For this review, take the finished solid that the model builds, in its own axes (mm). Give positions to 0.01 mm unless a question says otherwise; leave off trailing zeros. Loops run counter-clockwise (first coordinate to the right, second up) from the corner with the lowest first, then second, coordinate; pieces in that order, holes last.
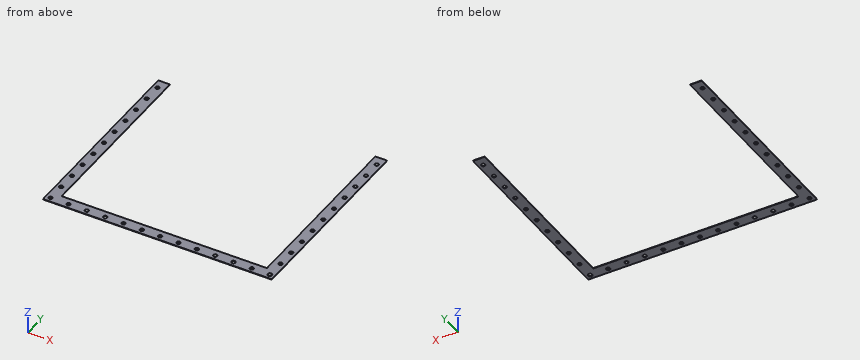
```python
from build123d import *

# Parameters (mm, degrees)
SKETCH1_R           = 12
SKETCH1_R_2         = 13.848900056
BOSS_EXTRUDE1_DEPTH = 3


with BuildPart() as part:
    # Sketch1 → Boss-Extrude1 (new body)
    # profile 1 of 2: a face of its own
    with BuildSketch(Plane.XY):
        with BuildLine():
            Line((7.821297611, 64.305720246), (-66.178702389, 64.305720246))
            Line((-66.178702389, 64.305720246), (-66.178702389, -1185.694279754))
            Line((-66.178702389, -1185.694279754), (657.821297611, -1185.694279754))
            Line((657.821297611, -1185.694279754), (657.821297611, -1167.694279754))
            ThreePointArc((657.821297611, -1167.694279754), (645.821297611, -1155.694279754), (657.821297611, -1143.694279754))
            Line((657.821297611, -1143.694279754), (657.821297611, -1111.694279754))
            Line((657.821297611, -1111.694279754), (7.821297611, -1111.694279754))
            Line((7.821297611, -1111.694279754), (7.821297611, 64.305720246))
        make_face()
        with Locations((-36.178702389, -1155.694279754)):
            Circle(SKETCH1_R, mode=Mode.SUBTRACT)
        with Locations((77.821297611, -1155.694279754)):
            Circle(SKETCH1_R, mode=Mode.SUBTRACT)
        with Locations((-36.178702389, -1039.694279754)):
            Circle(SKETCH1_R, mode=Mode.SUBTRACT)
        with Locations((193.821297611, -1155.694279754)):
            Circle(SKETCH1_R, mode=Mode.SUBTRACT)
        with Locations((-36.178702389, -923.694279754)):
            Circle(SKETCH1_R, mode=Mode.SUBTRACT)
        with Locations((309.821297611, -1155.694279754)):
            Circle(SKETCH1_R, mode=Mode.SUBTRACT)
        with Locations((425.821297611, -1155.694279754)):
            Circle(SKETCH1_R, mode=Mode.SUBTRACT)
        with Locations((541.821297611, -1155.694279754)):
            Circle(SKETCH1_R, mode=Mode.SUBTRACT)
        with Locations((-36.178702389, -807.694279754)):
            Circle(SKETCH1_R, mode=Mode.SUBTRACT)
        with Locations((-36.178702389, -691.694279754)):
            Circle(SKETCH1_R, mode=Mode.SUBTRACT)
        with Locations((-36.178702389, -575.694279754)):
            Circle(SKETCH1_R, mode=Mode.SUBTRACT)
        with Locations((-36.178702389, -459.694279754)):
            Circle(SKETCH1_R, mode=Mode.SUBTRACT)
        with Locations((-36.178702389, -343.694279754)):
            Circle(SKETCH1_R, mode=Mode.SUBTRACT)
        with Locations((-36.178702389, -227.694279754)):
            Circle(SKETCH1_R, mode=Mode.SUBTRACT)
        with Locations((-36.178702389, -111.694279754)):
            Circle(SKETCH1_R, mode=Mode.SUBTRACT)
        with Locations((-36.178702389, 4.305720246)):
            Circle(SKETCH1_R, mode=Mode.SUBTRACT)
    # profile 2 of 2: a face of its own
    with BuildSketch(Plane.XY):
        with BuildLine():
            Line((657.821297611, -1167.694279754), (657.821297611, -1185.694279754))
            Line((657.821297611, -1185.694279754), (1381.821297611, -1185.694279754))
            Line((1381.821297611, -1185.694279754), (1381.821297611, 64.305720246))
            Line((1381.821297611, 64.305720246), (1307.821297611, 64.305720246))
            Line((1307.821297611, 64.305720246), (1307.821297611, -1111.694279754))
            Line((1307.821297611, -1111.694279754), (657.821297611, -1111.694279754))
            Line((657.821297611, -1111.694279754), (657.821297611, -1143.694279754))
            ThreePointArc((657.821297611, -1143.694279754), (666.306578985, -1147.20899838), (669.821297611, -1155.694279754))
            ThreePointArc((669.821297611, -1155.694279754), (666.306578985, -1164.179561128), (657.821297611, -1167.694279754))
        make_face()
        with Locations((773.821297611, -1155.694279754)):
            Circle(SKETCH1_R, mode=Mode.SUBTRACT)
        with Locations((889.821297611, -1155.694279754)):
            Circle(SKETCH1_R, mode=Mode.SUBTRACT)
        with Locations((1005.821297611, -1155.694279754)):
            Circle(SKETCH1_R, mode=Mode.SUBTRACT)
        with Locations((1121.821297611, -1155.694279754)):
            Circle(SKETCH1_R, mode=Mode.SUBTRACT)
        with Locations((1237.821297611, -1155.694279754)):
            Circle(SKETCH1_R, mode=Mode.SUBTRACT)
        with Locations((1351.821297611, -1155.694279754)):
            Circle(SKETCH1_R_2, mode=Mode.SUBTRACT)
        with Locations((1351.821297611, -1039.694279754)):
            Circle(SKETCH1_R, mode=Mode.SUBTRACT)
        with Locations((1351.821297611, -923.694279754)):
            Circle(SKETCH1_R, mode=Mode.SUBTRACT)
        with Locations((1351.821297611, -807.694279754)):
            Circle(SKETCH1_R, mode=Mode.SUBTRACT)
        with Locations((1351.821297611, -691.694279754)):
            Circle(SKETCH1_R, mode=Mode.SUBTRACT)
        with Locations((1351.821297611, -575.694279754)):
            Circle(SKETCH1_R, mode=Mode.SUBTRACT)
        with Locations((1351.821297611, -459.694279754)):
            Circle(SKETCH1_R, mode=Mode.SUBTRACT)
        with Locations((1351.821297611, -343.694279754)):
            Circle(SKETCH1_R, mode=Mode.SUBTRACT)
        with Locations((1351.821297611, -227.694279754)):
            Circle(SKETCH1_R, mode=Mode.SUBTRACT)
        with Locations((1351.821297611, -111.694279754)):
            Circle(SKETCH1_R, mode=Mode.SUBTRACT)
        with Locations((1351.821297611, 4.305720246)):
            Circle(SKETCH1_R, mode=Mode.SUBTRACT)
    extrude(amount=BOSS_EXTRUDE1_DEPTH)


solid = part.part
```
Q1. Consider section A-A on y = -67. Give the boundary of the cut face in (x, z), plus the area to 3 significant figures.
Answers:
outline: (-66.18, 0) - (7.82, 0) - (7.82, 3) - (-66.18, 3) - close; (1307.82, 0) - (1381.82, 0) - (1381.82, 3) - (1307.82, 3) - close
area: 444 mm2
Q2. For pin 1 Ø1 at (x, z) = (346.5, 2) entering from +Y, flat-tipped, find the tip position at first contact; note if it passes through.
Answers:
pin 1: stops at y = -1111.69
Q3. For probe 1 along X at (y, z) = (-323, 1); probe 2 along X at (y, z) = (-217.5, 1); probe 3 along Y at (x, z) = (23, 1.5), list the stretches that pass through material, from the lowest coordinate up.
Answers:
probe 1: x = -66.18 to 7.82, 1307.82 to 1381.82
probe 2: x = -66.18 to -42.51, -29.85 to 7.82, 1307.82 to 1345.49, 1358.15 to 1381.82
probe 3: y = -1185.69 to -1111.69
Q4. Consider section C-C on x = 1081.5. Give the boundary of the cut face in (y, z), plus the area to 3 significant figures.
Answers:
outline: (-1185.69, 0) - (-1111.69, 0) - (-1111.69, 3) - (-1185.69, 3) - close
area: 222 mm2
Q5. Consider section B-B on z = 1.1. Count the separate pieces of the cut face and the enclosed holes in it, plus the area to 3 significant figures.
Answers:
separate pieces: 1
enclosed holes: 33
area: 266,000 mm2
